Read the model definition and answer for the solid it produces. Units are mm, in the model's axes. A direction names the side the tool comes from. Coordinates: 2 decimals unless noted, no trailing zeros. Write each loop counter-clockwise with the first axis right and the second up, starting at its lowest first coordinate (ties: lowest second). Pieces come first, ordered by that corner, then holes. Notation, with made-up numbers: (40.25, 23.25) -> (96.25, 23.25) arc R35 ccw to (96.25, 56.25) -> close; hole circle Ø6 at (-10, 70). An arc over 180 degrees is marked (long way). One line per item, written item: value. Start each with the question number.
1. For faces 4 (the flat face through (19.5, -9.5, -0.1)), 5 (the cylindrical face through (-16.87, -3.36, 5.83)), 6 (the flat face through (7, 7, -4)), determine the directions among +Z, -Z, +X, -X, +Y, -Y from which every point of the face is accessible in a straight line to the end or side of a thin tool.
2. Consider line 1 along Y through (x, z) = (14, -3.25); line 2 along X through (y, z) = (-1.25, -7); line 3 along X through (y, z) = (4.5, -6.25). Determine where each line is inside the solid, lowest interval first.
3. Find section D-D, the plane x = -14. Write down the section's boundary in (y, z).
4. Find section A-A, the plane z = -6.75. Write down the section's boundary in (x, y), and give its area (3 significant figures).
5. Find section B-B, the plane x = 6. Write down the section's boundary in (y, z).
6. Given P1, Ø7, axis at x = 14, y = 6, coming from the +Z side; P2, Ø3.5, axis at x = 14, y = -6, coming from the +Z side; P3, Ø1, axis at x = -0.5, y = -6, coming from the -Z side, each flat-ended and moving along its own axis, determine where each tip first touches the part or whether it passes through.
7. For a pull along X with two mould halves and no side action, classify faces 1 (the flat face through (0, -10, 2)), 2 (the flat face through (19.5, 9.5, 0.1)), 3 (the flat face through (-12, -8, 3.6)) as pulls with the +X half, pulls with the -X half, needs draft (parallel to the pull), parting line crosses it, or undercut.
8. Find section C-C, the plane z = 5.75. Write down the section's boundary in (x, y).
```python
from build123d import *

# Parameters (mm, degrees)
SKETCH_1_W                   = 40
SKETCH_1_H                   = 20
EXTRUDE_1_DEPTH              = 8
CHAMFER_1_SIZE               = 1
HOLE_WIZARD_15_0_15_1_D      = 15
HOLE_WIZARD_15_0_15_1_DEPTH  = 20
CUT_EXTRUDE_2_DEPTH          = 8
HOLE_WIZARD_M4_3_D           = 4.5
HOLE_WIZARD_M4_3_CBORE_D     = 7.8
HOLE_WIZARD_M4_3_CBORE_DEPTH = 4.4


with BuildPart() as part:
    # 草图1 → 凸台-拉伸1 (new, symmetric)
    with BuildSketch(Plane.XY):
        Rectangle(SKETCH_1_W, SKETCH_1_H)
    extrude(amount=EXTRUDE_1_DEPTH, both=True)

    # 倒角1
    chamfer_1_edges = [part.edges().sort_by_distance(p)[0] for p in [
        (20, -10, 0),
        (-20, -10, 0),
        (-20, 10, 0),
        (20, 10, 0),
    ]]
    chamfer(chamfer_1_edges, length=CHAMFER_1_SIZE)

    # Ø15.0 (15) 直径孔1
    with Locations(Plane.XY.offset(8)):
        with Locations((0, 2)):
            Hole(HOLE_WIZARD_15_0_15_1_D / 2, depth=HOLE_WIZARD_15_0_15_1_DEPTH)

    # 草图6 → 切除-拉伸2 (cut)
    with BuildSketch(Plane(origin=(0, 0, -8), x_dir=(-1, 0, 0), z_dir=(0, 0, -1))):
        Polygon((-7, -14.985571338), (-7, 13.139303821), (7, 13.139303821), (7, -15.772038878), align=None)
    extrude(amount=-CUT_EXTRUDE_2_DEPTH, mode=Mode.SUBTRACT)

    # M4 六角凹头螺钉的柱形沉头孔3 (through all)
    with Locations(Plane.XY.offset(8)):
        with Locations((0, 0), (14, 6), (-14, -6), (-14, 6), (14, -6)):
            CounterBoreHole(HOLE_WIZARD_M4_3_D / 2, HOLE_WIZARD_M4_3_CBORE_D / 2, HOLE_WIZARD_M4_3_CBORE_DEPTH)


solid = part.part
```
Answer block:
1. face 4: +Z, -Z, +X, -Y
1. face 5: +Z
1. face 6: -Z, +Y, -Y
2. line 1: y = -10 to -8.25, -3.75 to 3.75, 8.25 to 10
2. line 2: x = -20 to -7, 7 to 20
2. line 3: x = -20 to -15.68, -12.32 to -7.07, 7.07 to 12.32, 15.68 to 20
3. outline: (-10, -8) -> (-8.25, -8) -> (-8.25, 3.6) -> (-9.9, 3.6) -> (-9.9, 8) -> (-10, 8) -> close; (-3.75, -8) -> (3.75, -8) -> (3.75, 3.6) -> (2.1, 3.6) -> (2.1, 8) -> (-2.1, 8) -> (-2.1, 3.6) -> (-3.75, 3.6) -> close; (8.25, -8) -> (10, -8) -> (10, 8) -> (9.9, 8) -> (9.9, 3.6) -> (8.25, 3.6) -> close
4. outline: (-20, -9) -> (-19, -10) -> (-7, -10) -> (-7, -0.69) arc R7.5 cw to (-7, 4.69) -> (-7, 10) -> (-19, 10) -> (-20, 9) -> close; (7, -10) -> (19, -10) -> (20, -9) -> (20, 9) -> (19, 10) -> (7, 10) -> (7, 4.69) arc R7.5 cw to (7, -0.69) -> close; hole circle Ø4.5 at (-14, -6); hole circle Ø4.5 at (-14, 6); hole circle Ø4.5 at (14, -6); hole circle Ø4.5 at (14, 6)
4. area: 451 mm2
5. outline: (-10, 0) -> (-2.5, 0) -> (-2.5, 8) -> (-10, 8) -> close; (6.5, 0) -> (10, 0) -> (10, 8) -> (6.5, 8) -> close
6. P1: stops at z = 3.6
6. P2: passes through
6. P3: stops at z = 0
7. face 1: needs draft
7. face 2: pulls with the +X half
7. face 3: undercut
8. outline: (-20, -9) -> (-19, -10) -> (19, -10) -> (20, -9) -> (20, 9) -> (19, 10) -> (-19, 10) -> (-20, 9) -> close; hole circle Ø7.8 at (-14, -6); hole circle Ø7.8 at (-14, 6); hole circle Ø15 at (0, 2); hole circle Ø7.8 at (14, -6); hole circle Ø7.8 at (14, 6)
